from build123d import *

# Parameters (mm, degrees)
BASE_PLATE_55X7_DEPTH         = 3.5
FRONT_NOTCH_SKETCH_W          = 13
FRONT_NOTCH_SKETCH_H          = 9.412383513
FRONT_NOTCH_13X6_5_DEPTH      = 32.38621781
UPRIGHT_A_SKETCH_W            = 10
UPRIGHT_A_SKETCH_H            = 32
UPRIGHT_A_10X32_DEPTH         = 14.717156
UPRIGHT_B_SKETCH_W            = 10
UPRIGHT_B_SKETCH_H            = 32
UPRIGHT_B_10X32_DEPTH         = 14.717156
UPRIGHT_A_HOLE_SKETCH_R       = 3.5
UPRIGHT_A_HOLE_DEPTH          = 39.016443898
INFILL_BOSS_SKETCH_W          = 13
INFILL_BOSS_SKETCH_H          = 32
INFILL_BOSS_DEPTH             = 14.717156
REAR_NOTCH_SKETCH_W           = 13
REAR_NOTCH_SKETCH_H           = 13
REAR_NOTCH_13X6_5_DEPTH       = 43.250380835
SLOT_CUT_SKETCH_W             = 9
SLOT_CUT_SKETCH_H             = 15
SLOT_CUT_DEPTH                = 43.250380835
UPRIGHT_B_HOLE_SKETCH_R       = 3.5
UPRIGHT_B_HOLE_DEPTH          = 54.030651577
FLANGE_PROFILE_CUT_A_SKETCH_W = 2
FLANGE_PROFILE_CUT_A_SKETCH_H = 25
FLANGE_PROFILE_CUT_A_DEPTH    = 43.250380835
FLANGE_PROFILE_CUT_B_DEPTH    = 43.250380835


with BuildPart() as part:
    # Base Plate Sketch → Base Plate 55x7 (new, symmetric)
    with BuildSketch(Plane(origin=(0, 0, 0), x_dir=(1, 0, 0), z_dir=(0, 1, 0))):
        Polygon((-20.480974443, -6.717155582), (19.519025557, -6.717155582), (27.5, -2), (27.5, 8), (-27.5, 8), (-27.5, -2), align=None)
    extrude(amount=BASE_PLATE_55X7_DEPTH, both=True)

    # Front Notch Sketch → Front Notch 13x6.5 (cut, through all)
    with BuildSketch(Plane.XY.offset(6.717155582)):
        with Locations((0, -0.276834809)):
            Rectangle(FRONT_NOTCH_SKETCH_W, FRONT_NOTCH_SKETCH_H)
    extrude(amount=-FRONT_NOTCH_13X6_5_DEPTH, mode=Mode.SUBTRACT)


with BuildPart() as front_notch_13x6_5_piece_1:
    # of the separate pieces the step leaves, piece 1, a body of its own (front_notch_13x6_5_pieces)
    add(part.part.solids().sort_by_distance((-20.480974443, 3.5, 6.717155582))[0])

    # Upright A Sketch → Upright A 10x32 (add)
    with BuildSketch(Plane.XY.offset(6.717155582)):
        with Locations((-11.5, 12.5)):
            Rectangle(UPRIGHT_A_SKETCH_W, UPRIGHT_A_SKETCH_H)
    extrude(amount=-UPRIGHT_A_10X32_DEPTH)


with BuildPart() as front_notch_13x6_5_piece_2:
    # of the separate pieces the step leaves, piece 2, a body of its own (front_notch_13x6_5_pieces)
    add(part.part.solids().sort_by_distance((6.5, 3.5, 6.717155582))[0])

    # Upright B Sketch → Upright B 10x32 (add)
    with BuildSketch(Plane.XY.offset(6.717155582)):
        with Locations((11.5, 12.5)):
            Rectangle(UPRIGHT_B_SKETCH_W, UPRIGHT_B_SKETCH_H)
    extrude(amount=-UPRIGHT_B_10X32_DEPTH)


with BuildPart() as upright_a_hole_tool:
    # Upright A Hole Sketch → Upright A Hole (new, through all)
    with BuildSketch(Plane(origin=(0, 3.5, 0), x_dir=(1, 0, 0), z_dir=(0, 1, 0))):
        with Locations(Location((-22, 3, 0), (0, 0, 270))):
            Circle(UPRIGHT_A_HOLE_SKETCH_R)
        with Locations(Location((22, 3, 0), (0, 0, 270))):
            Circle(UPRIGHT_A_HOLE_SKETCH_R)
    extrude(amount=-UPRIGHT_A_HOLE_DEPTH)


with BuildPart() as front_notch_13x6_5_piece_1_1:
    add(front_notch_13x6_5_piece_1.part)

    # Upright A Hole: cut by upright_a_hole_tool
    add(upright_a_hole_tool.part, mode=Mode.SUBTRACT)



with BuildPart() as front_notch_13x6_5_piece_2_1:
    add(front_notch_13x6_5_piece_2.part)

    # Upright A Hole: cut by upright_a_hole_tool
    add(upright_a_hole_tool.part, mode=Mode.SUBTRACT)


with BuildPart() as front_notch_13x6_5_piece_1_2:
    add(front_notch_13x6_5_piece_1_1.part)

    add(front_notch_13x6_5_piece_2_1.part)  # Infill Boss merges Front Notch 13x6.5 piece 2
    # Infill Boss Sketch → Infill Boss (add, through all)
    with BuildSketch(Plane.XY.offset(6.717155582)):
        with Locations((0, 12.5)):
            Rectangle(INFILL_BOSS_SKETCH_W, INFILL_BOSS_SKETCH_H)
    extrude(amount=-INFILL_BOSS_DEPTH)

    # Rear Notch Sketch → Rear Notch 13x6.5 (cut, through all)
    with BuildSketch(Plane.XY.offset(6.717155582)):
        with Locations((0, 3)):
            Rectangle(REAR_NOTCH_SKETCH_W, REAR_NOTCH_SKETCH_H)
    extrude(amount=-REAR_NOTCH_13X6_5_DEPTH, mode=Mode.SUBTRACT)

    # Slot Cut Sketch → Slot Cut (cut, through all)
    with BuildSketch(Plane.XY.offset(6.717155582)):
        with Locations((0, 21)):
            Rectangle(SLOT_CUT_SKETCH_W, SLOT_CUT_SKETCH_H)
    extrude(amount=-SLOT_CUT_DEPTH, mode=Mode.SUBTRACT)

    # Upright B Hole Sketch → Upright B Hole (cut, through all)
    with BuildSketch(Plane(origin=(16.5, 0, 0), x_dir=(0, 0, -1), z_dir=(1, 0, 0))):
        with Locations((0.641422209, 22.5)):
            Circle(UPRIGHT_B_HOLE_SKETCH_R)
    extrude(amount=-UPRIGHT_B_HOLE_DEPTH, mode=Mode.SUBTRACT)

    # Flange Profile Cut A Sketch → Flange Profile Cut A (cut, through all)
    with BuildSketch(Plane.XY.offset(6.717155582)):
        with Locations((15.5, 16)):
            Rectangle(FLANGE_PROFILE_CUT_A_SKETCH_W, FLANGE_PROFILE_CUT_A_SKETCH_H)
    extrude(amount=-FLANGE_PROFILE_CUT_A_DEPTH, mode=Mode.SUBTRACT)

    # Flange Profile Cut B Sketch → Flange Profile Cut B (cut, through all)
    with BuildSketch(Plane.XY.offset(6.717155582)):
        Polygon((-14.5, 3.425354954), (-14.5, 28.5), (-16.5, 28.5), (-16.5, 3.5), align=None)
    extrude(amount=-FLANGE_PROFILE_CUT_B_DEPTH, mode=Mode.SUBTRACT)


solid = front_notch_13x6_5_piece_1_2.part
For this review, take the finished solid that the model builds, in its own axes (mm). A direction names the side the tool comes from. Coordinates: 2 decimals unless noted, no trailing zeros. Write each loop counter-clockwise with the first axis right and the second up, starting at its lowest first coordinate (ties: lowest second). Pieces come first, ordered by that corner, then holes. Notation, with made-up numbers: (52, -35) -> (75, -35) arc R12 cw to (75, -12) -> close; hole circle Ø8 at (-26.5, -7.5). An arc over 180 degrees is marked (long way). Write each question's results on one line, items separated by ' | '. Start each with the question number.
1) Consider section A-A (y = 7). Write out the cut boundary in (x, z).
2) Consider section B-B (x = -12). Write out the cut boundary in (y, z).
3) Consider section C-C (z = -0.5). Give the number of separate pieces and of enclosed holes in the cut face, plus the area to 3 significant figures.
4) Wall thickness on L1, parallel to X at y = -0.75, z = -3; L2, parallel to X at y = 1.5, z = -5; L3, parallel to X at y = 21.5, z = -4.75: over which ranges is each line inside the solid? List them lowest first. Write a range as [from, to].
5) The part is to be moulded in two halves that separate along Y. For faces 1 (the face through (25.47, 0.05, -3.46)), 2 (the face through (9.57, 25.97, -0.19)), 3 (the face through (-22, 3.5, 1)), say which applies: +Y half, -Y half, draft (parallel to the pull), parting line (faces both ways), or undercut.
6) Consider section D-D (y = 22.5). Write out the cut boundary in (x, z).
7) Insertion check: pin 1 (7.5 mm diameter, centred on y = 19.5, z = -3.5, fed in from -X); pin 2 (8 mm diameter, centred on x = 21, z = 3, fed in from +Y); pin 3 (6 mm diameter, centred on y = 17.5, z = -5.5, fed in from +X). Each pin has a flat end and moves straight along its axis. Give the tip position at first contact, or say it passes through.
8) For faces 4 (the face through (0, 9.5, -1)), 5 (the face through (4.5, 19, 1)), 6 (the face through (-10, 28.5, -1)), 7 (the face through (14.5, 16, -1)), list the 3-axis set-ups (+Z, -Z, +X, -X, +Y, -Y) from which the entire face can be reached by the end or side of a thin tool; tool diameter is ignored.
Geometry says:
1) outline: (-14.5, -8) -> (-6.5, -8) -> (-6.5, 6.72) -> (-14.5, 6.72) -> close; (6.5, -8) -> (14.5, -8) -> (14.5, 6.72) -> (6.5, 6.72) -> close
2) outline: (-3.5, -8) -> (28.5, -8) -> (28.5, 6.72) -> (-3.5, 6.72) -> close; hole circle Ø7 at (22.5, -0.64)
3) separate pieces: 5 | enclosed holes: 0 | area: 597 mm^2
4) L1: [-27.5, -25.5], [-18.5, -6.5], [6.5, 18.5], [25.5, 27.5] | L2: [-27.5, -24.87], [-19.13, -6.5], [6.5, 19.13], [24.87, 27.5] | L3: [-14.5, -4.5], [4.5, 14.5]
5) face 1: draft | face 2: undercut | face 3: +Y half
6) outline: (-14.5, -8) -> (-4.5, -8) -> (-4.5, -4.14) -> (-14.5, -4.14) -> close; (-14.5, 2.86) -> (-4.5, 2.86) -> (-4.5, 6.72) -> (-14.5, 6.72) -> close; (4.5, -8) -> (14.5, -8) -> (14.5, -4.14) -> (4.5, -4.14) -> close; (4.5, 2.86) -> (14.5, 2.86) -> (14.5, 6.72) -> (4.5, 6.72) -> close
7) pin 1: x = -14.5 | pin 2: y = 3.5 | pin 3: x = 14.5
8) face 4: +Z, -Z, -Y | face 5: +Z, -Z, +Y | face 6: +Z, -Z, +X, -X, +Y | face 7: +Z, -Z, +X, +Y
